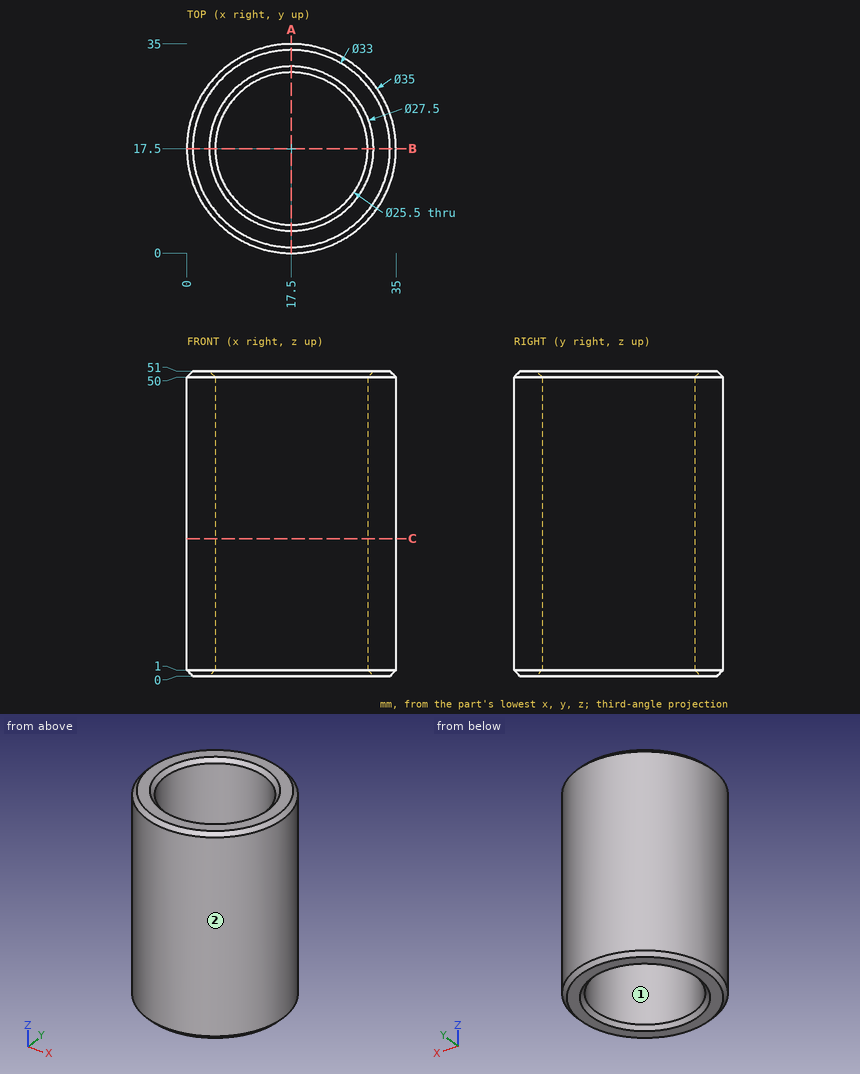
Geometry check sheet. Reference: drawing and pictorial views, mm from the part's lowest x, y, z. Coordinates: 2 decimals unless noted, no trailing zeros. Write each loop counter-clockwise with the first axis right and the second up, starting at its lowest first coordinate (ties: lowest second). Pieces come first, ordered by that corner, then holes. Notation, with made-up numbers: (76, 20.5) - (90, 20.5) arc R9 ccw to (90, 30.5) - close; hole circle Ø7 at (-25.75, 17.25). An arc over 180 degrees is marked (long way). Write item = value, one per line.
Q1. Material ranges on L1, parallel to Y at x = 17, z = 32; L2, parallel to Y at x = 13.5, z = 12, recorded low to high. Write a range as from..to.
Answer:
L1 = 0.01..4.76, 30.24..34.99
L2 = 0.46..5.39, 29.61..34.54
Q2. Mould release check, pull along Y, two halves, no side actions. Record for the marked faces 1 and 2: released by +Y, released by -Y, zero draft, split by the parting line, or undercut.
Answer:
face_1 = undercut
face_2 = split by the parting line
Q3. Cross-section at C-C (z = 23). Enter the section's corners in (x, y).
Answer:
outline = circle Ø35 at (17.5, 17.5); hole circle Ø25.5 at (17.5, 17.5)
Q4. Go/stop test with flat-tipped pins: pin 1 Ø5 at (y, z) = (13.5, 37.5) entering from +X; pin 2 Ø6 at (y, z) = (4.5, 17.5) entering from +X; pin 3 Ø6 at (y, z) = (5, 29.5) entering from +X; pin 4 Ø1 at (x, y) = (20.5, 28) entering from +Z. Record where each tip stops, or that it passes through.
Answer:
pin_1 = 34.94
pin_2 = 31.86
pin_3 = 32.2
pin_4 = through
Q5. Cross-section at A-A (x = 17.5). Enter the section's corners in (y, z).
Answer:
outline = (0, 1) - (1, 0) - (3.75, 0) - (4.75, 1) - (4.75, 50) - (3.75, 51) - (1, 51) - (0, 50) - close; (30.25, 1) - (31.25, 0) - (34, 0) - (35, 1) - (35, 50) - (34, 51) - (31.25, 51) - (30.25, 50) - close
